Source: CAD feature listing. Evaluate the final solid. Frame: model axes, mm. Give positions to 0.01 mm unless a question says otherwise; leave off trailing zeros. Order: outer loops, then holes, each group sorted by start corner. A loop starts at its lowest first (then second) coordinate and runs counter-clockwise, first axis right, second up. Notation, with made-up numbers: M 67.5,67.25 L 122.5,67.25 A17 ccw 122.5,77.25 Z; hole C 7,-35 d4. An arc over 180 degrees is marked long. Use CSV: the item, a comma, the result in double quotes. Start each with the question number.
Item 1: Section query A-A on x = 60. Return loops of the section in (y, z).
Item 2: Ray query, probe 1 along X at (y, z) = (2, -25); probe 2 along X at (y, z) = (-1.75, 75); probe 3 along Z at (x, y) = (-41.25, 1.75). Return the intervals inside material, ascending. Write a range as from..to.
Item 3: Section query C-C on x = 0. Return loops of the section in (y, z).
Item 4: Section query B-B on z = -75. Return loops of the section in (x, y), and give its area (3 significant figures).
Item 5: Section query D-D on z = 83. Return loops of the section in (x, y).
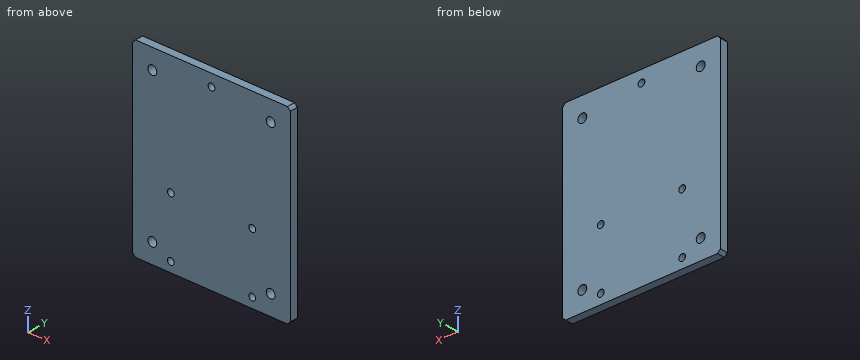
from build123d import *

# Parameters (mm, degrees)
SKETCH_1_W            = 160
SKETCH_1_H            = 190
EXTRUDE_1_DEPTH       = 4
CHAMFER_1_SIZE        = 3
HOLE_WIZARD_9_0_9_1_D = 9
HOLE_WIZARD_M8_2_D    = 6.8
HOLE_WIZARD_M8_1_D    = 6.8


with BuildPart() as part:
    # 草图1 → 凸台-拉伸1 (new, symmetric)
    with BuildSketch(Plane(origin=(0, 0, 0), x_dir=(1, 0, 0), z_dir=(0, 1, 0))):
        Rectangle(SKETCH_1_W, SKETCH_1_H)
    extrude(amount=EXTRUDE_1_DEPTH, both=True)

    # 倒角1
    chamfer_1_edges = [part.edges().sort_by_distance(p)[0] for p in [
        (80, 0, 95),
        (-80, 0, 95),
        (-80, 0, -95),
        (80, 0, -95),
    ]]
    chamfer(chamfer_1_edges, length=CHAMFER_1_SIZE)

    # Ø9.0 (9) 直径孔1 (through all)
    with Locations(Plane(origin=(0, -4, 0), x_dir=(-1, 0, 0), z_dir=(0, -1, 0))):
        with Locations((-60, -75), (60, -75), (60, 75), (-60, 75)):
            Hole(HOLE_WIZARD_9_0_9_1_D / 2)

    # M8 螺纹孔2 (through all)
    with Locations(Plane(origin=(0, -4, 0), x_dir=(-1, 0, 0), z_dir=(0, -1, 0))):
        with Locations((-41.25, 25), (-41.25, 85), (41.25, 85), (41.25, 25)):
            Hole(HOLE_WIZARD_M8_2_D / 2)

    # M8 螺纹孔1 (through all)
    with Locations(Plane(origin=(0, -4, 0), x_dir=(-1, 0, 0), z_dir=(0, -1, 0))):
        with Locations((0, -83)):
            Hole(HOLE_WIZARD_M8_1_D / 2)


solid = part.part
Verdict:
1,outline,"M -4,-95 L 4,-95 L 4,-79.5 L -4,-79.5 Z; M -4,-70.5 L 4,-70.5 L 4,70.5 L -4,70.5 Z; M -4,79.5 L 4,79.5 L 4,95 L -4,95 Z"
2,probe 1,"-80..-44.65, -37.85..37.85, 44.65..80"
2,probe 2,"-80..-64.5, -55.5..55.5, 64.5..80"
2,probe 3,"-95..-88.4, -81.6..-28.4, -21.6..95"
3,outline,"M -4,-95 L 4,-95 L 4,79.6 L -4,79.6 Z; M -4,86.4 L 4,86.4 L 4,95 L -4,95 Z"
4,outline,"M -80,-4 L -64.5,-4 L -64.5,4 L -80,4 Z; M -55.5,-4 L 55.5,-4 L 55.5,4 L -55.5,4 Z; M 64.5,-4 L 80,-4 L 80,4 L 64.5,4 Z"
4,area,"1,140 mm2"
5,outline,"M -80,-4 L -3.4,-4 L -3.4,4 L -80,4 Z; M 3.4,-4 L 80,-4 L 80,4 L 3.4,4 Z"
